For this review, take the finished solid that the model builds, in its own axes (mm). A direction names the side the tool comes from. Coordinates: 2 decimals unless noted, no trailing zeros. Write each loop counter-clockwise with the first axis right and the second up, starting at its lowest first coordinate (ties: lowest second). Pieces come first, ordered by that corner, then holes.
```python
from build123d import *

# Parameters (mm, degrees)
BASE_BLOCK_SKETCH_W     = 64
BASE_BLOCK_SKETCH_H     = 75
BASE_BLOCK_DEPTH        = 20
CLAMP_LUG_A_SKETCH_W    = 12
CLAMP_LUG_A_SKETCH_H    = 75
CLAMP_LUG_A_DEPTH       = 22
CLAMP_LUG_B_SKETCH_W    = 12
CLAMP_LUG_B_SKETCH_H    = 75
CLAMP_LUG_B_DEPTH       = 22
ADJUSTMENT_SLOT_A_DEPTH = 101.463923873
ADJUSTMENT_SLOT_B_DEPTH = 101.463923873
MOUNTING_TAB_SKETCH_R   = 8
MOUNTING_TAB_DEPTH      = 10
BACK_WALL_CUT_SKETCH_R  = 8
BACK_WALL_CUT_DEPTH     = 156.128978595
LUG_A_EDGE_FILLET_R12_R = 12
LUG_B_EDGE_FILLET_R12_R = 12


with BuildPart() as part:
    # Base Block Sketch → Base Block (new body)
    with BuildSketch(Plane.XY):
        with Locations((32, 37.5)):
            Rectangle(BASE_BLOCK_SKETCH_W, BASE_BLOCK_SKETCH_H)
    extrude(amount=BASE_BLOCK_DEPTH)

    # Clamp Lug A Sketch → Clamp Lug A (add)
    with BuildSketch(Plane.XY.offset(20)):
        with Locations((6, 37.5)):
            Rectangle(CLAMP_LUG_A_SKETCH_W, CLAMP_LUG_A_SKETCH_H)
    extrude(amount=CLAMP_LUG_A_DEPTH)

    # Clamp Lug B Sketch → Clamp Lug B (add)
    with BuildSketch(Plane.XY.offset(20)):
        with Locations((58, 37.5)):
            Rectangle(CLAMP_LUG_B_SKETCH_W, CLAMP_LUG_B_SKETCH_H)
    extrude(amount=CLAMP_LUG_B_DEPTH)

    # Adjustment Slot A Sketch → Adjustment Slot A (cut, through all)
    with BuildSketch(Plane(origin=(12, 0, 0), x_dir=(0, 0, -1), z_dir=(1, 0, 0))):
        with BuildLine():
            Line((-37, 15.5), (-37, 59.5))
            ThreePointArc((-37, 59.5), (-31, 65.5), (-25, 59.5))
            Line((-25, 59.5), (-25, 15.5))
            ThreePointArc((-25, 15.5), (-31, 9.5), (-37, 15.5))
        make_face()
    extrude(amount=-ADJUSTMENT_SLOT_A_DEPTH, mode=Mode.SUBTRACT)

    # Adjustment Slot B Sketch → Adjustment Slot B (cut, through all)
    with BuildSketch(Plane.ZY.offset(-52)):
        with BuildLine():
            Line((25, 15.5), (25, 59.5))
            ThreePointArc((25, 59.5), (31, 65.5), (37, 59.5))
            Line((37, 59.5), (37, 15.5))
            ThreePointArc((37, 15.5), (31, 9.5), (25, 15.5))
        make_face()
    extrude(amount=-ADJUSTMENT_SLOT_B_DEPTH, mode=Mode.SUBTRACT)

    # Mounting Tab Sketch → Mounting Tab (add)
    with BuildSketch(Plane.XY):
        with BuildLine():
            Line((114, 57.5), (76, 57.5))
            ThreePointArc((76, 57.5), (67.514718626, 61.014718626), (64, 69.5))
            Line((64, 69.5), (64, 5.5))
            ThreePointArc((64, 5.5), (67.514718626, 13.985281374), (76, 17.5))
            Line((76, 17.5), (114, 17.5))
            ThreePointArc((114, 17.5), (134, 37.5), (114, 57.5))
        make_face()
        with Locations((114, 37.5)):
            Circle(MOUNTING_TAB_SKETCH_R, mode=Mode.SUBTRACT)
    extrude(amount=MOUNTING_TAB_DEPTH)

    # Back Wall Cut Sketch → Back Wall Cut (cut, through all)
    with BuildSketch(Plane.XY.offset(20)):
        with Locations((32, 59.5)):
            Circle(BACK_WALL_CUT_SKETCH_R)
        with Locations((32, 15.5)):
            Circle(BACK_WALL_CUT_SKETCH_R)
    extrude(amount=-BACK_WALL_CUT_DEPTH, mode=Mode.SUBTRACT)

    # Lug A Edge Fillet R12
    lug_a_edge_fillet_r12_edges = [part.edges().sort_by_distance(p)[0] for p in [
        (6, 0, 42),
        (6, 75, 42),
    ]]
    fillet(lug_a_edge_fillet_r12_edges, radius=LUG_A_EDGE_FILLET_R12_R)

    # Lug B Edge Fillet R12
    lug_b_edge_fillet_r12_edges = [part.edges().sort_by_distance(p)[0] for p in [
        (58, 0, 42),
        (58, 75, 42),
    ]]
    fillet(lug_b_edge_fillet_r12_edges, radius=LUG_B_EDGE_FILLET_R12_R)


solid = part.part
```
Q1. For probe 1 along Y at (x, z) = (32, 7); probe 2 along X at (y, z) = (37, 8); probe 3 along Y at (x, z) = (114, 5.75), list the stretches that pass through material, from the lowest coordinate up.
Ans:
probe 1: y = 0 to 7.5, 23.5 to 51.5, 67.5 to 75
probe 2: x = 0 to 106.02, 121.98 to 133.99
probe 3: y = 17.5 to 29.5, 45.5 to 57.5
Q2. Add section B-B (y = 37.5). State the section outline as (x, z) points, then the cut area to 3 significant figures.
Ans:
outline: (0, 0) - (106, 0) - (106, 10) - (64, 10) - (64, 25) - (52, 25) - (52, 20) - (12, 20) - (12, 25) - (0, 25) - close; (0, 37) - (12, 37) - (12, 42) - (0, 42) - close; (52, 37) - (64, 37) - (64, 42) - (52, 42) - close; (122, 0) - (134, 0) - (134, 10) - (122, 10) - close
area: 2,060 mm2
Q3. Add section C-C (z = 4). State the section outline as (x, y) points, then the cut area to 3 significant figures.
Ans:
outline: (0, 0) - (64, 0) - (64, 5.5) arc R12 cw to (76, 17.5) - (114, 17.5) arc R20 ccw to (114, 57.5) - (76, 57.5) arc R12 cw to (64, 69.5) - (64, 75) - (0, 75) - close; hole circle Ø16 at (32, 15.5); hole circle Ø16 at (32, 59.5); hole circle Ø16 at (114, 37.5)
area: 6,890 mm2
Q4. Add section A-A (x = 32). State the section outline as (y, z) points.
Ans:
outline: (0, 0) - (7.5, 0) - (7.5, 20) - (0, 20) - close; (23.5, 0) - (51.5, 0) - (51.5, 20) - (23.5, 20) - close; (67.5, 0) - (75, 0) - (75, 20) - (67.5, 20) - close
Q5. Add section D-D (x = 120). State the section outline as (y, z) points.
Ans:
outline: (18.42, 0) - (32.21, 0) - (32.21, 10) - (18.42, 10) - close; (42.79, 0) - (56.58, 0) - (56.58, 10) - (42.79, 10) - close
Q6. Clearance check with flat-ended pins moving along their axes: pin 1 Ø12.5 at (y, z) = (33.5, 20.5) entering from +X; pin 2 Ø11 at (x, z) = (92.5, 4.5) entering from +Y; pin 3 Ø12 at (x, y) = (38.5, 19) entering from +Z; pin 4 Ø4 at (x, y) = (29.5, 10.5) entering from +Z. State where each tip first meets the part, or that it passes through.
Ans:
pin 1: stops at x = 64
pin 2: stops at y = 57.5
pin 3: stops at z = 20
pin 4: passes through
Q7. Tool access review of faces 1 (the flat face through (91, 38, 10)), 2 (the flat face through (58, 37, 25)), 3 (the flat face through (95, 17.5, 5)), 4 (the flat face through (95, 57.5, 5)): name each direction out of +Z, -Z, +X, -X, +Y, -Y from which nothing blocks a thin tool from reaching the whole face with its end or side.
Ans:
face 1: +Z, +X, +Y, -Y
face 2: +X, -X
face 3: +Z, -Z, +X, -Y
face 4: +Z, -Z, +X, +Y
Q8. Draft analysis for pull direction Z (two halves, no side actions). For faces 5 (the cylindrical face through (6.1, 9.5, 30.9)), 6 (the cylindrical face through (121.63, 39.9, 4.93)), 7 (the flat face through (32, 38, 20)), state which applies: +Z half, -Z half, draft (parallel to the pull), parting line (faces both ways), or undercut.
Ans:
face 5: undercut
face 6: draft
face 7: +Z half
